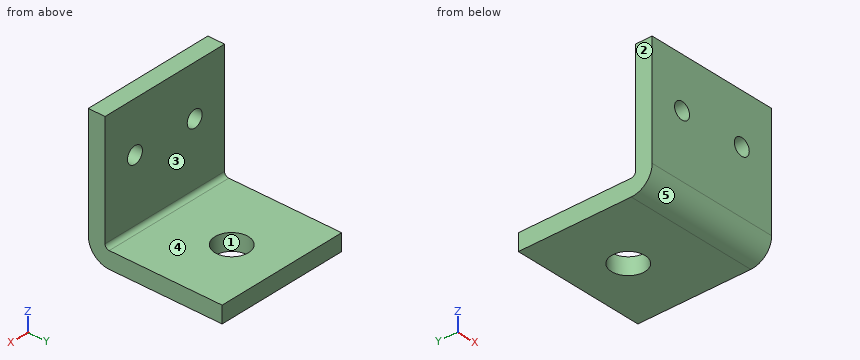
```python
from build123d import *

# Parameters (mm, degrees)
BOSS_EXTRUDE1_DEPTH = 40
SKETCH2_R           = 5
CUT_EXTRUDE1_DEPTH  = 40
SKETCH3_R           = 2.5
CUT_EXTRUDE2_DEPTH  = 40


with BuildPart() as part:
    # Sketch1 → Boss-Extrude1 (new body)
    with BuildSketch(Plane(origin=(0, 0, 0), x_dir=(0, 0, -1), z_dir=(1, 0, 0))):
        with BuildLine():
            Line((11.805555556, 25.625), (11.805555556, -8.125))
            ThreePointArc((11.805555556, -8.125), (11.439439032, -9.008883476), (10.555555556, -9.375))
            Line((10.555555556, -9.375), (-23.194444444, -9.375))
            Line((-23.194444444, -9.375), (-23.194444444, -14.375))
            Line((-23.194444444, -14.375), (10.555555556, -14.375))
            ThreePointArc((10.555555556, -14.375), (14.974972938, -12.544417382), (16.805555556, -8.125))
            Line((16.805555556, -8.125), (16.805555556, 25.625))
            Line((16.805555556, 25.625), (11.805555556, 25.625))
        make_face()
    extrude(amount=-BOSS_EXTRUDE1_DEPTH)

    # Sketch2 → Cut-Extrude1 (cut)
    with BuildSketch(Plane.XY.offset(-11.805555556)):
        with Locations((-20, 10.625)):
            Circle(SKETCH2_R)
    extrude(amount=-CUT_EXTRUDE1_DEPTH, mode=Mode.SUBTRACT)

    # Sketch3 → Cut-Extrude2 (cut)
    with BuildSketch(Plane(origin=(0, -9.375, 0), x_dir=(1, 0, 0), z_dir=(0, 1, 0))):
        with Locations(Location((-30, -8.194444444, 0), (0, 0, 270))):
            Circle(SKETCH3_R)
        with Locations(Location((-10, -8.194444444, 0), (0, 0, 270))):
            Circle(SKETCH3_R)
    extrude(amount=-CUT_EXTRUDE2_DEPTH, mode=Mode.SUBTRACT)


solid = part.part
```
The listing builds one solid part. Answer for the finished solid, in the listing's coordinates (mm). Face numbers are marked on the shaded views. A direction names the side the tool comes from. Give positions to 0.01 mm unless a question says otherwise; leave off trailing zeros. Order: outer loops, then holes, each group sorted by start corner. A loop starts at its lowest first (then second) coordinate and runs counter-clockwise, first axis right, second up. Notation, with made-up numbers: (11.5, 35.5) - (57.5, 35.5) arc R15 ccw to (57.5, 41.5) - close; hole circle Ø9 at (17, 2). An arc over 180 degrees is marked (long way). Use one line per item in the form item = value. Start each with the question number.
(1) A cutting plane is placed at B-B, the plane z = 10. Write down the section's boundary in (x, y) (3 decimals).
(2) The mould has two halves that part along X. Classify the marked faces 1, 2 and 3: released by +X, released by -X, zero draft, split by the parting line, or undercut.
(3) For the marked faces 4 and 5, determine the directions among +Z, -Z, +X, -X, +Y, -Y from which every point of the face is accessible in a straight line to the end or side of a thin tool.
(4) A cutting plane is placed at C-C, the plane x = -35.5. Write down the section's boundary in (y, z) (3 decimals).
(5) Consider line 1 (Y direction, x = -5.5, z = 8) (3 decimals); line 2 (Z direction, x = -25, y = -3); line 3 (Y direction, x = -20, z = -13) (3 decimals). Determine where each line is inside the solid, lowest interval first. Write a range as from..to.
(6) A cutting plane is placed at D-D, the plane z = 4. Write down the section's boundary in (x, y) (3 decimals).
(7) Flat-ended cylindrical pins translate along their axes: pin 1 Ø12 at (x, z) = (-15.5, -11) entering from +Y (3 decimals); pin 2 Ø8 at (x, y) = (-20, 10.625) entering from -Z; pin 3 Ø10 at (x, z) = (-19.5, 10) entering from +Y (3 decimals); pin 4 Ø10 at (x, y) = (-28, 10) entering from +Z. Find the tip coordinate at first contact, or state that the pin passes through.
(8) A cutting plane is placed at A-A, the plane x = -10. Write down the section's boundary in (y, z) (3 decimals), then the cut area to 3 significant figures.
Ans:
q1.outline = (-40, -14.375) - (-31.729, -14.375) - (-31.729, -9.375) - (-40, -9.375) - close; (-28.271, -14.375) - (-11.729, -14.375) - (-11.729, -9.375) - (-28.271, -9.375) - close; (-8.271, -14.375) - (0, -14.375) - (0, -9.375) - (-8.271, -9.375) - close
q2.face_1 = undercut
q2.face_2 = released by -X
q2.face_3 = zero draft
q3.face_4 = +Z, +X, -X, +Y
q3.face_5 = -Z, +X, -X, -Y
q4.outline = (-14.375, -10.556) arc R6.25 ccw to (-8.125, -16.806) - (25.625, -16.806) - (25.625, -11.806) - (-8.125, -11.806) arc R1.25 cw to (-9.375, -10.556) - (-9.375, 23.194) - (-14.375, 23.194) - close
q5.line_1 = -14.375..-9.375
q5.line_2 = -16.81..-11.81
q5.line_3 = -13.877..5.625, 15.625..25.625
q6.outline = (-40, -14.375) - (0, -14.375) - (0, -9.375) - (-40, -9.375) - close
q7.pin_1 = 25.625
q7.pin_2 = through
q7.pin_3 = -9.375
q7.pin_4 = -11.81
q8.outline = (-14.375, -10.556) arc R6.25 ccw to (-8.125, -16.806) - (25.625, -16.806) - (25.625, -11.806) - (-8.125, -11.806) arc R1.25 cw to (-9.375, -10.556) - (-9.375, 5.694) - (-14.375, 5.694) - close; (-14.375, 10.694) - (-9.375, 10.694) - (-9.375, 23.194) - (-14.375, 23.194) - close
q8.area = 342 mm^2
